Input: part model. Units: mm. Frame: model coordinates. Face numbers are marked on the shaded views. A direction names the side the tool comes from. Give positions to 0.01 mm unless a question says otherwise; leave off trailing zeros. Loops run counter-clockwise (first coordinate to the right, second up) from the corner with the lowest first, then second, coordinate; pieces in that order, holes last.
from build123d import *

# Parameters (mm, degrees)
SKETCH_1_W          = 12.5
SKETCH_1_H          = 6
EXTRUDE_1_DEPTH     = 7.5
SKETCH_2_W          = 11.342894438
SKETCH_2_H          = 4.477163802
SKETCH_2_R          = 0.480353021
SKETCH_2_R_2        = 0.517183851
SKETCH_2_R_3        = 0.582724364
SKETCH_2_R_4        = 0.500500501
CUT_EXTRUDE_1_DEPTH = 5
SKETCH_3_W          = 0.643352529
SKETCH_3_H          = 1.364086891
EXTRUDE_2_DEPTH     = 8


with BuildPart() as part:
    # 草图1 → 拉伸1 (new body)
    with BuildSketch(Plane.XY):
        with Locations((5.032975889, 1.613598403)):
            Rectangle(SKETCH_1_W, SKETCH_1_H)
    extrude(amount=EXTRUDE_1_DEPTH)

    # 草图2 → 切除-拉伸1 (cut)
    with BuildSketch(Plane(origin=(0, 0, 0), x_dir=(-1, 0, 0), z_dir=(0, 0, -1))):
        with Locations((-5.104708636, 1.729550555)):
            Rectangle(SKETCH_2_W, SKETCH_2_H)
        with Locations((-7.986319653, 2.191858525)):
            Circle(SKETCH_2_R, mode=Mode.SUBTRACT)
        with Locations((-6.334668001, 2.191858525)):
            Circle(SKETCH_2_R_2, mode=Mode.SUBTRACT)
        with Locations((-4.299299299, 2.191858525)):
            Circle(SKETCH_2_R_3, mode=Mode.SUBTRACT)
        with Locations((-2.230563897, 2.191858525)):
            Circle(SKETCH_2_R_4, mode=Mode.SUBTRACT)
    extrude(amount=-CUT_EXTRUDE_1_DEPTH, mode=Mode.SUBTRACT)

    # 草图3 → 拉伸2 (add)
    with BuildSketch(Plane(origin=(0, 4.613598403, 4.886401597), x_dir=(1, 0, 0), z_dir=(0, -1, 0))):
        with Locations((6.598992375, 2.512158379)):
            Rectangle(SKETCH_3_W, SKETCH_3_H)
        with Locations((9.598992375, 2.512158379)):
            Rectangle(SKETCH_3_W, SKETCH_3_H)
        with Locations((3.598992375, 2.512158379)):
            Rectangle(SKETCH_3_W, SKETCH_3_H)
        with Locations((0.598992376, 2.512158379)):
            Rectangle(SKETCH_3_W, SKETCH_3_H)
    extrude(amount=EXTRUDE_2_DEPTH)


solid = part.part
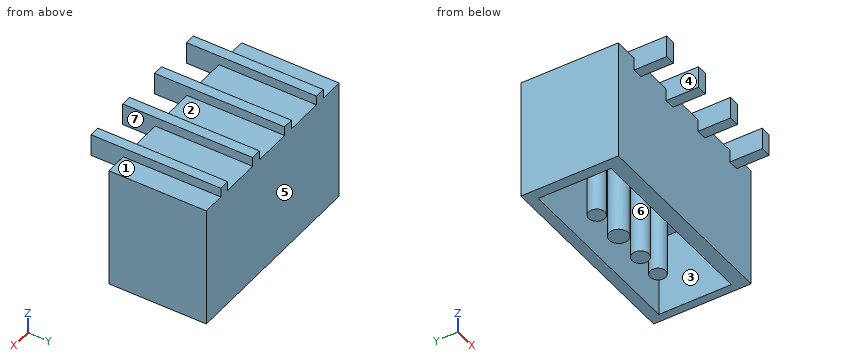
(1) Cut plane C-C (y = -0.75). Return the cut outline in (x, z), and give its area (3 significant figures).
Values follow:
outline: (-1.22, 0) - (11.28, 0) - (11.28, 7.5) - (9.92, 7.5) - (9.92, 8.08) - (9.28, 8.08) - (9.28, 7.5) - (6.92, 7.5) - (6.92, 8.08) - (6.28, 8.08) - (6.28, 7.5) - (3.92, 7.5) - (3.92, 8.08) - (3.28, 8.08) - (3.28, 7.5) - (0.92, 7.5) - (0.92, 8.08) - (0.28, 8.08) - (0.28, 7.5) - (-1.22, 7.5) - close
area: 95.2 mm2
(2) Ray query, probe 1 along X at (y, z) = (3.5, 3.25); probe 2 along Y at (x, z) = (-0.25, 4); probe 3 along Z at (x, y) = (5.25, 2.75). Return the intervals inside material, ascending.
Values follow:
probe 1: x = -1.22 to -0.57, 10.78 to 11.28
probe 2: y = -1.39 to -0.51, 3.97 to 4.61
probe 3: z = 5 to 7.5
(3) Cut plane A-A (x = 10.25). Return the cut outline in (y, z).
Values follow:
outline: (-1.39, 0) - (-0.51, 0) - (-0.51, 5) - (3.97, 5) - (3.97, 0) - (4.61, 0) - (4.61, 7.5) - (-1.39, 7.5) - close
(4) Mould query, pull axis Y, two halves, no side actions, for the marked faces 5, 6 and 7. Classes: +Y half, -Y half, draft (parallel to the pull), parting line (faces both ways), or undercut.
Values follow:
face 5: +Y half
face 6: undercut
face 7: draft
(5) Cut plane D-D (z = 7.25). Return the cut outline in (x, y), and give its area (3 significant figures).
Values follow:
outline: (-1.22, -1.39) - (0.28, -1.39) - (0.28, -3.39) - (0.92, -3.39) - (0.92, -1.39) - (3.28, -1.39) - (3.28, -3.39) - (3.92, -3.39) - (3.92, -1.39) - (6.28, -1.39) - (6.28, -3.39) - (6.92, -3.39) - (6.92, -1.39) - (9.28, -1.39) - (9.28, -3.39) - (9.92, -3.39) - (9.92, -1.39) - (11.28, -1.39) - (11.28, 4.61) - (-1.22, 4.61) - close
area: 80.1 mm2
(6) Cut plane B-B (z = 1). Return the cut outline in (x, y).
Values follow:
outline: (-1.22, -1.39) - (11.28, -1.39) - (11.28, 4.61) - (-1.22, 4.61) - close; circle Ø1 at (2.23, 2.19); circle Ø1.17 at (4.3, 2.19); circle Ø1.03 at (6.33, 2.19); circle Ø0.96 at (7.99, 2.19); hole (-0.57, -0.51) - (10.78, -0.51) - (10.78, 3.97) - (-0.57, 3.97) - close
(7) Reachability of the marked faces 1, 2, 3 and 4 from +Z, -Z, +X, -X, +Y, -Y: full face, straight path, thin tool, end or side. Return the list, or none.
Values follow:
face 1: +Z, +X, +Y, -Y
face 2: +Z, +Y, -Y
face 3: -Z
face 4: +Z, -Y
(8) Pin query (flat end, axial travel): pin 1 Ø0.7 at (x, y) = (6.5, -2.5) entering from -Z. Return the tip coordinate at first contact, or that it passes through.
Values follow:
pin 1: stops at z = 6.72
